Could you check a few things on this drawing? It's one solid part, dimensions in mm from its lowest x, y, z. A direction names the side the tool comes from. Round coordinates to 2 decimals unless told otherwise and drop trailing zeros. Use a Markdown table: item, result. Add a question column.
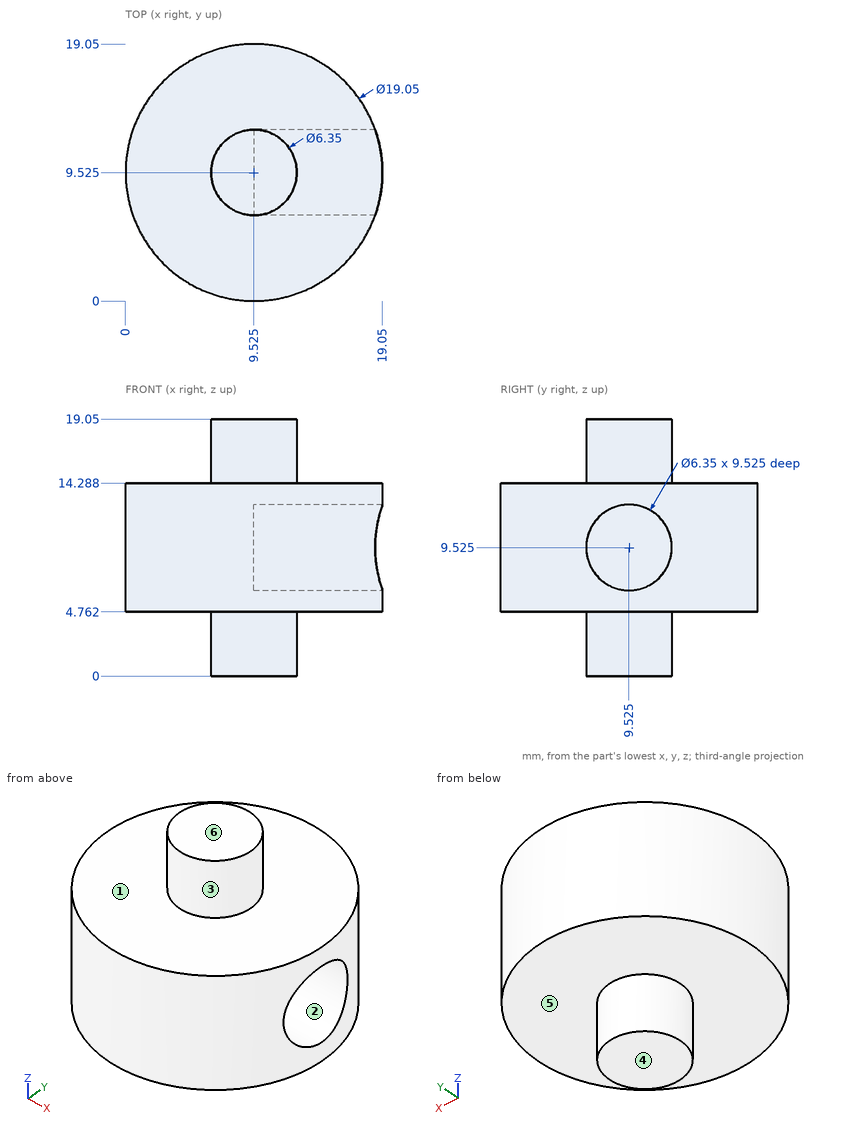
(1) I'm going to push flat-ended pins straight in: pin 1 (5.5 mm diameter, centred on x = 5, y = 7.5, fed in from +Z); pin 2 (1.5 mm diameter, centred on x = 13.5, y = 8.5, fed in from -Z); pin 3 (2 mm diameter, centred on y = 17, z = 6.5, fed in from -X); pin 4 (2 mm diameter, centred on x = 5, z = 4, fed in from +Y) (1 decimal). Where does each tip first touch, or does it pass through?
(2) If I drill on probe 1 along Z at (x, y) = (14.25, 4.5); probe 2 along Y at (x, z) = (3.5, 7); probe 3 along X at (y, z) = (7.5, 16), over which ranges is the centre line in solid material (lowest first)? Write a range as [from, to].
(3) On a 3-axis mill with a long thin cutter (end or side, diameter ignored), from which of +Z, -Z, +X, -X, +Y, -Y can I reach the whole of each face in a straight line? I mean the marked faces 5 and 6. Say none if no direction works.
(4) Thinking about a two-plate mould opening in Z: for the marked faces 1, 2, 3 and 4, which applies, released by +Z, released by -Z, zero draft, split by the parting line, or undercut?
Results below:
| question | item | result |
|---|---|---|
| 1 | pin 1 | stops at z = 19.05 |
| 1 | pin 2 | stops at z = 4.76 |
| 1 | pin 3 | stops at x = 2.54 |
| 1 | pin 4 | stops at y = 18.2 |
| 2 | probe 1 | z = [4.76, 14.29] |
| 2 | probe 2 | y = [2.15, 16.9] |
| 2 | probe 3 | x = [7.08, 11.97] |
| 3 | face 5 | -Z |
| 3 | face 6 | +Z, +X, -X, +Y, -Y |
| 4 | face 1 | released by +Z |
| 4 | face 2 | undercut |
| 4 | face 3 | zero draft |
| 4 | face 4 | released by -Z |
